```python
from build123d import *

# Parameters (mm, degrees)
SKETCH1_R           = 5
BOSS_EXTRUDE1_DEPTH = 5
CUT_EXTRUDE1_DEPTH  = 10


with BuildPart() as part:
    # Sketch1 → Boss-Extrude1 (new, symmetric)
    with BuildSketch(Plane(origin=(0, 0, 0), x_dir=(1, 0, 0), z_dir=(0, 1, 0))):
        with BuildLine():
            Line((0, 12.5), (150, 12.5))
            ThreePointArc((150, 12.5), (162.5, 0), (150, -12.5))
            Line((150, -12.5), (0, -12.5))
            ThreePointArc((0, -12.5), (-12.5, 0), (0, 12.5))
        make_face()
        with Locations(Location((0, 0, 0), (0, 0, 270))):
            Circle(SKETCH1_R, mode=Mode.SUBTRACT)
        with Locations(Location((150, 0, 0), (0, 0, 270))):
            Circle(SKETCH1_R, mode=Mode.SUBTRACT)
    extrude(amount=BOSS_EXTRUDE1_DEPTH, both=True)

    # Sketch2 → Cut-Extrude1 (cut)
    with BuildSketch(Plane(origin=(0, 5, 0), x_dir=(1, 0, 0), z_dir=(0, 1, 0))):
        with BuildLine():
            Line((25, 5), (125, 5))
            ThreePointArc((125, 5), (130, 0), (125, -5))
            Line((125, -5), (25, -5))
            ThreePointArc((25, -5), (20, 0), (25, 5))
        make_face()
    extrude(amount=-CUT_EXTRUDE1_DEPTH, mode=Mode.SUBTRACT)


solid = part.part
```
The listing builds one solid part. Answer for the finished solid, in the listing's coordinates (mm). A direction names the side the tool comes from. Give positions to 0.01 mm unless a question says otherwise; leave off trailing zeros. Loops run counter-clockwise (first coordinate to the right, second up) from the corner with the lowest first, then second, coordinate; pieces in that order, holes last. Notation, with made-up numbers: M -34.5,49 L 10.5,49 A9 cw 10.5,57 Z; hole C 24,-23 d10. An arc over 180 degrees is marked long. One line per item, written item: value.
Q1. Flat-ended cylindrical pins translate along their axes: P1, Ø3, axis at y = -2.5, z = -4.5, coming from the +X side; P2, Ø2, axis at y = 1.5, z = -2.5, coming from the +X side. Find the tip coordinate at first contact, or state that the pin passes through.
Working result:
P1: stops at x = 162.13
P2: stops at x = 162.41
Q2. A cutting plane is placed at B-B on x = 53.5. Determine the outline of the cut face in (y, z).
Working result:
outline: M -5,-12.5 L 5,-12.5 L 5,-5 L -5,-5 Z; M -5,5 L 5,5 L 5,12.5 L -5,12.5 Z
Q3. Determine the mould class of faces 3 (the face through (145.564, -0.07, 2.307)), 4 (the face through (20, 0, 0)), 5 (the face through (74, 0, -12.5)), 6 (the face through (76, -5, -6)) for opening direction Z: +Z half, -Z half, draft (parallel to the pull), parting line (faces both ways), or undercut.
Working result:
face 3: undercut
face 4: undercut
face 5: -Z half
face 6: draft
Q4. For faces 1 (the face through (-12.497, 0.07, 0.275)), 2 (the face through (74, 0, -5)), determine the directions among +Z, -Z, +X, -X, +Y, -Y from which every point of the face is accessible in a straight line to the end or side of a thin tool.
Working result:
face 1: -X, +Y, -Y
face 2: +Y, -Y
Q5. A cutting plane is placed at D-D on z = 7.75. Determine the outline of the cut face in (x, y), then the cut area to 3 significant figures.
Working result:
outline: M -9.81,-5 L 159.81,-5 L 159.81,5 L -9.81,5 Z
area: 1,700 mm^2
Q6. A cutting plane is placed at A-A on y = -0.25. Determine the outline of the cut face in (x, z).
Working result:
outline: M 0,-12.5 L 150,-12.5 A12.5 ccw 150,12.5 L 0,12.5 A12.5 ccw Z; hole C 0,0 d10; hole M 25,-5 L 125,-5 A5 ccw 125,5 L 25,5 A5 ccw Z; hole C 150,0 d10
Q7. Find the intervals of material crossed by line 1 (X direction, y = 1, z = 0); line 2 (Z direction, x = 118, y = 4.5); line 3 (X direction, y = 0.75, z = -3), in increasing order. Write a range as from..to.
Working result:
line 1: x = -12.5..-5, 5..20, 130..145, 155..162.5
line 2: z = -12.5..-5, 5..12.5
line 3: x = -12.13..-4, 4..21, 129..146, 154..162.13
Q8. A cutting plane is placed at C-C on z = 0. Determine the outline of the cut face in (x, y), then the cut area to 3 significant figures.
Working result:
outline: M -12.5,-5 L -5,-5 L -5,5 L -12.5,5 Z; M 5,-5 L 20,-5 L 20,5 L 5,5 Z; M 130,-5 L 145,-5 L 145,5 L 130,5 Z; M 155,-5 L 162.5,-5 L 162.5,5 L 155,5 Z
area: 450 mm^2
